```python
from build123d import *

# Parameters (mm, degrees)
SKETCH_1_R          = 11
EXTRUDE_1_DEPTH     = 4
SKETCH_2_R          = 8.5
EXTRUDE_2_DEPTH     = 12.5
EXTRUDE_START       = 8
SKETCH_9_R          = 11
EXTRUDE_3_DEPTH     = 8
M10X1_25_1_D        = 8.8
CUT_EXTRUDE_2_DEPTH = 33.46921619
SKETCH_10_W         = 1
SKETCH_10_H         = 12.5
CUT_EXTRUDE_3_DEPTH = 24.5


with BuildPart() as part:
    # 草图1 → 凸台-拉伸1 (new, symmetric)
    with BuildSketch(Plane(origin=(0, 0, 0), x_dir=(1, 0, 0), z_dir=(0, 1, 0))):
        with Locations(Location((0, 0, 0), (0, 0, 270))):
            Circle(SKETCH_1_R)
    extrude(amount=EXTRUDE_1_DEPTH, both=True)

    # 草图2 → 凸台-拉伸2 (add)
    with BuildSketch(Plane(origin=(0, 4, 0), x_dir=(1, 0, 0), z_dir=(0, 1, 0))):
        with Locations(Location((0, 0, 0), (0, 0, 270))):
            Circle(SKETCH_2_R)
    extrude(amount=EXTRUDE_2_DEPTH)

    # 草图9 → 凸台-拉伸3 (add)
    with BuildSketch(Plane(origin=(0, 16.5, 0), x_dir=(1, 0, 0), z_dir=(0, 1, 0)).offset(EXTRUDE_START)):
        with Locations(Location((0, 0, 0), (0, 0, 270))):
            Circle(SKETCH_9_R)
    extrude(amount=-EXTRUDE_3_DEPTH)

    # M10x1.25 螺纹孔1 (through all)
    with Locations(Plane(origin=(0, -4, 0), x_dir=(-1, 0, 0), z_dir=(0, -1, 0))):
        with Locations((0, 0)):
            Hole(M10X1_25_1_D / 2)

    # 草图6 → 切除-拉伸2 (cut, through all)
    with BuildSketch(Plane.XZ.offset(4)):
        with BuildLine():
            Line((-4.582575695, 10), (4.582575695, 10))
            ThreePointArc((4.582575695, 10), (0, 11), (-4.582575695, 10))
        make_face()
        with BuildLine():
            Line((-4.582575695, -10), (4.582575695, -10))
            ThreePointArc((4.582575695, -10), (0, -11), (-4.582575695, -10))
        make_face()
    extrude(amount=-CUT_EXTRUDE_2_DEPTH, mode=Mode.SUBTRACT)

    # 草图10 → 切除-拉伸3 (cut, symmetric)
    with BuildSketch(Plane.XY):
        with Locations((-8, 10.25)):
            Rectangle(SKETCH_10_W, SKETCH_10_H)
        with Locations((8, 10.25)):
            Rectangle(SKETCH_10_W, SKETCH_10_H)
    extrude(amount=CUT_EXTRUDE_3_DEPTH, both=True, mode=Mode.SUBTRACT)


solid = part.part
```
Verification items for the finished model (mm, model axes). A direction names the side the tool comes from. Round coordinates to 2 decimals unless told otherwise and drop trailing zeros. Write each loop counter-clockwise with the first axis right and the second up, starting at its lowest first coordinate (ties: lowest second). Pieces come first, ordered by that corner, then holes.
1. Section check C-C on y = 3.5. Enter the section's corners in (x, z), plus the area to 3 significant figures.
2. Gauge pin test, flat ends, axial feed: P1, Ø2.5, axis at y = 12.5, z = 1, coming from the +X side; P2, Ø6, axis at x = -6.5, y = 9, coming from the +Z side; P3, Ø8, axis at x = 7.5, y = 13.5, coming from the -Z side; P4, Ø6, axis at x = -8.5, z = -7.5, coming from the +Y side. Record the tip position at first contact, or that the pin passes through.
3. Section check B-B on z = 0. Enter the section's corners in (x, y), plus the area to 3 significant figures.
4. Section check A-A on x = 0. Enter the section's corners in (y, z), plus the area to 3 significant figures.
5. Section check D-D on x = 7. Enter the section's corners in (y, z), plus the area to 3 significant figures.
6. Access from +Z, -Z, +X, -X, +Y, -Y to the whole of each face (thin tool, end or side, straight path). Record for faces 4 (the flat face through (-7.5, 10, 0)), 5 (the flat face through (8, 16.5, 0)), 6 (the flat face through (7.5, 10, 0)), 7 (the cylindrical face through (0.1, 10.2, -8.5)).
7. Scan lines: L1, parallel to X at y = -2.5, z = 0.25; L2, parallel to Z at x = 0, y = 9.75; L3, parallel to Y at x = -4.25, z = -8. Record each from-to range of solid material in increasing order.
8. Draft check along Y on faces 1 (the cylindrical face through (11, 21, 0)), 2 (the flat face through (8, 4, 0)), 3 (the flat face through (0, 24.5, -5)). Enter one of: +Y half, -Y half, draft (parallel to the pull), parting line (faces both ways), or undercut.
Answer:
1. outline: (-4.58, -10) - (4.58, -10) arc R11 ccw to (4.58, 10) - (-4.58, 10) arc R11 ccw to start; hole circle Ø8.8 at (0, 0)
1. area: 307 mm2
2. P1: stops at x = 7.5
2. P2: stops at z = 7.75
2. P3: stops at z = -9.87
2. P4: stops at y = 24.5
3. outline: (-11, -4) - (-4.4, -4) - (-4.4, 24.5) - (-11, 24.5) - (-11, 16.5) - (-7.5, 16.5) - (-7.5, 4) - (-11, 4) - close; (4.4, -4) - (11, -4) - (11, 4) - (7.5, 4) - (7.5, 16.5) - (11, 16.5) - (11, 24.5) - (4.4, 24.5) - close
3. area: 289 mm2
4. outline: (-4, -10) - (4, -10) - (4, -8.5) - (16.5, -8.5) - (16.5, -10) - (24.5, -10) - (24.5, -4.4) - (-4, -4.4) - close; (-4, 4.4) - (24.5, 4.4) - (24.5, 10) - (16.5, 10) - (16.5, 8.5) - (4, 8.5) - (4, 10) - (-4, 10) - close
4. area: 282 mm2
5. outline: (-4, -8.49) - (4, -8.49) - (4, -4.82) - (16.5, -4.82) - (16.5, -8.49) - (24.5, -8.49) - (24.5, 8.49) - (16.5, 8.49) - (16.5, 4.82) - (4, 4.82) - (4, 8.49) - (-4, 8.49) - close
5. area: 392 mm2
6. face 4: +Z, -Z, -X
6. face 5: none
6. face 6: +Z, -Z, +X
6. face 7: -Z
7. L1: x = -11 to -4.39, 4.39 to 11
7. L2: z = -8.5 to -4.4, 4.4 to 8.5
7. L3: y = -4 to 4, 16.5 to 24.5
8. face 1: draft
8. face 2: undercut
8. face 3: +Y half
